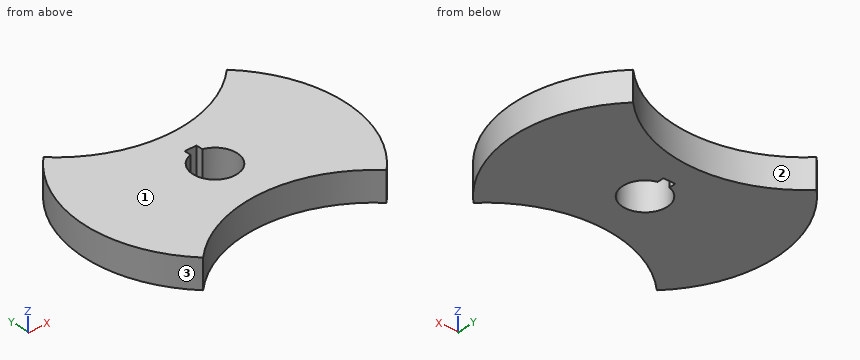
```python
from build123d import *

# Parameters (mm, degrees)
EXTRUDE_1_DEPTH     = 20
CUT_EXTRUDE_1_DEPTH = 110.617516848


with BuildPart() as part:
    # 草图1 → 凸台-拉伸1 (new body)
    with BuildSketch(Plane.XY):
        with BuildLine():
            ThreePointArc((-62.225396744, 62.225396744), (-88, 0), (-62.225396744, -62.225396744))
            ThreePointArc((-62.225396744, -62.225396744), (0, -36.450793489), (62.225396744, -62.225396744))
            ThreePointArc((62.225396744, -62.225396744), (88, 0), (62.225396744, 62.225396744))
            ThreePointArc((62.225396744, 62.225396744), (0, 36.450793489), (-62.225396744, 62.225396744))
        make_face()
    extrude(amount=EXTRUDE_1_DEPTH)

    # 草图2 → 切除-拉伸1 (cut, through all)
    with BuildSketch(Plane.XY.offset(20)):
        with BuildLine():
            Line((-4, 19), (4, 19))
            Line((4, 19), (4, 14.456832295))
            ThreePointArc((4, 14.456832295), (0, -15), (-4, 14.456832295))
            Line((-4, 14.456832295), (-4, 19))
        make_face()
    extrude(amount=-CUT_EXTRUDE_1_DEPTH, mode=Mode.SUBTRACT)


solid = part.part
```
The model under review builds one solid part; all positions refer to its coordinate system, in mm. Face numbers are marked on the shaded views. Coordinates: 2 decimals unless noted, no trailing zeros. Write each loop counter-clockwise with the first axis right and the second up, starting at its lowest first coordinate (ties: lowest second). Pieces come first, ordered by that corner, then holes. Notation, with made-up numbers: (31, -17.5) -> (79, -17.5) arc R19 cw to (79, 7.5) -> close; hole circle Ø8 at (16.5, -37). An arc over 180 degrees is marked (long way). One line per item, written item: value. Start each with the question number.
Q1. The part is to be moulded in two halves that separate along X. For the marked faces 1, 2 and 3, say which applies: +X half, -X half, draft (parallel to the pull), parting line (faces both ways), or undercut.
Q2. Clearance check with flat-ended pins moving along their axes: P1, Ø9, axis at x = 2, z = 8, coming from the -Y side; P2, Ø10, axis at x = 65.5, z = 17.5, coming from the +Y side; P3, Ø5, axis at y = 18, z = 7, coming from the +X side; P4, Ø2.5, axis at y = 16.5, z = 5, coming from the -X side. State where each tip first meets the part, or that it passes through.
Q3. Add section D-D, the plane x = -57. Give the boundary of the cut face in (y, z), then the cut area to 3 significant figures.
Q4. Add section B-B, the plane y = 0. Give the boundary of the cut face in (x, z).
Q5. Add section C-C, the plane z = 9.5. Give the boundary of the cut face in (x, y).
Q6. To check wall thickness, follow probe 1 along Y at (x, z) = (0, 5.25); probe 2 along X at (y, z) = (0, 16.25); probe 3 along Y at (x, z) = (-11.5, 8.25). State the ranges of each line that lie inside material, in increasing order.
Q7. Add section A-A, the plane x = 0. Give the boundary of the cut face in (y, z).
Response:
1. face 1: draft
1. face 2: undercut
1. face 3: -X half
2. P1: y = -36.69
2. P2: y = 62.23
2. P3: x = 86.62
2. P4: x = -86.67
3. outline: (-57.41, 0) -> (57.41, 0) -> (57.41, 20) -> (-57.41, 20) -> close
3. area: 2,300 mm²
4. outline: (-88, 0) -> (-15, 0) -> (-15, 20) -> (-88, 20) -> close; (15, 0) -> (88, 0) -> (88, 20) -> (15, 20) -> close
5. outline: (-62.23, -62.23) arc R88 cw to (62.23, -62.23) arc R88 ccw to (62.23, 62.23) arc R88 cw to (-62.23, 62.23) arc R88 ccw to start; hole (-4, 14.46) arc R15 ccw (long way) to (4, 14.46) -> (4, 19) -> (-4, 19) -> close
6. probe 1: -36.45 to -15, 19 to 36.45
6. probe 2: -88 to -15, 15 to 88
6. probe 3: -37.21 to -9.63, 9.63 to 37.21
7. outline: (-36.45, 0) -> (-15, 0) -> (-15, 20) -> (-36.45, 20) -> close; (19, 0) -> (36.45, 0) -> (36.45, 20) -> (19, 20) -> close
